```python
from build123d import *

# Parameters (mm, degrees)
SKETCH_2_R          = 11
CUT_EXTRUDE_1_DEPTH = 2
CUT_EXTRUDE_2_REACH = 196.342
SKETCH_3_R          = 5.5
SKETCH_4_R          = 5
CUT_EXTRUDE_3_DEPTH = 46


with BuildPart() as part:
    # 草图1 → 旋转1 (revolve)
    with BuildSketch(Plane.XY, mode=Mode.PRIVATE) as revolve_1_sk:
        with BuildLine():
            Line((65, 35), (57.5, 35))
            Line((57.5, 35), (57.5, 60))
            Line((57.5, 60), (100, 60))
            Line((100, 60), (100, 0))
            Line((100, 0), (130, 0))
            Line((130, 0), (130, -40))
            Line((130, -40), (87.5, -40))
            ThreePointArc((87.5, -40), (80.428932188, -42.928932188), (77.5, -50))
            Line((77.5, -50), (77.5, -65))
            Line((77.5, -65), (65, -65))
            Line((65, -65), (65, 35))
        make_face()
    revolve(revolve_1_sk.sketch.rotate(Axis((0, 133.6875, 0), (0, -1, 0)), 90), axis=Axis((0, 133.6875, 0), (0, -1, 0)))

    # 草图2 → 切除-拉伸1 (cut)
    with BuildSketch(Plane(origin=(0, 0, 0), x_dir=(1, 0, 0), z_dir=(0, 1, 0))):
        with Locations(Location((115, 0, 0), (0, 0, 270))):
            Circle(SKETCH_2_R)
        with Locations(Location((81.317279836, -81.317279836, 0), (0, 0, 270))):
            Circle(SKETCH_2_R)
        with Locations(Location((0, -115, 0), (0, 0, 270))):
            Circle(SKETCH_2_R)
        with Locations(Location((-81.317279836, -81.317279836, 0), (0, 0, 270))):
            Circle(SKETCH_2_R)
        with Locations(Location((-115, 0, 0), (0, 0, 270))):
            Circle(SKETCH_2_R)
        with Locations(Location((-81.317279836, 81.317279836, 0), (0, 0, 270))):
            Circle(SKETCH_2_R)
        with Locations(Location((0, 115, 0), (0, 0, 270))):
            Circle(SKETCH_2_R)
        with Locations(Location((81.317279836, 81.317279836, 0), (0, 0, 270))):
            Circle(SKETCH_2_R)
    extrude(amount=-CUT_EXTRUDE_1_DEPTH, mode=Mode.SUBTRACT)

    # 草图3 → 切除-拉伸2 (cut, up to next)
    with BuildSketch(Plane(origin=(0, -2, 0), x_dir=(1, 0, 0), z_dir=(0, 1, 0)), mode=Mode.PRIVATE) as cut_extrude_2_sk1:
        with Locations(Location((81.317279836, 81.317279836, 0), (0, 0, 270))):
            Circle(SKETCH_3_R)
    cut_extrude_2_tool1 = extrude(cut_extrude_2_sk1.sketch, amount=-CUT_EXTRUDE_2_REACH, mode=Mode.PRIVATE) & part.part
    # 草图3 → 切除-拉伸2 (cut, up to next)
    with BuildSketch(Plane(origin=(0, -2, 0), x_dir=(1, 0, 0), z_dir=(0, 1, 0)), mode=Mode.PRIVATE) as cut_extrude_2_sk2:
        with Locations(Location((115, 0, 0), (0, 0, 270))):
            Circle(SKETCH_3_R)
    cut_extrude_2_tool2 = extrude(cut_extrude_2_sk2.sketch, amount=-CUT_EXTRUDE_2_REACH, mode=Mode.PRIVATE) & part.part
    # 草图3 → 切除-拉伸2 (cut, up to next)
    with BuildSketch(Plane(origin=(0, -2, 0), x_dir=(1, 0, 0), z_dir=(0, 1, 0)), mode=Mode.PRIVATE) as cut_extrude_2_sk3:
        with Locations(Location((81.317279836, -81.317279836, 0), (0, 0, 270))):
            Circle(SKETCH_3_R)
    cut_extrude_2_tool3 = extrude(cut_extrude_2_sk3.sketch, amount=-CUT_EXTRUDE_2_REACH, mode=Mode.PRIVATE) & part.part
    # 草图3 → 切除-拉伸2 (cut, up to next)
    with BuildSketch(Plane(origin=(0, -2, 0), x_dir=(1, 0, 0), z_dir=(0, 1, 0)), mode=Mode.PRIVATE) as cut_extrude_2_sk4:
        with Locations(Location((0, -115, 0), (0, 0, 270))):
            Circle(SKETCH_3_R)
    cut_extrude_2_tool4 = extrude(cut_extrude_2_sk4.sketch, amount=-CUT_EXTRUDE_2_REACH, mode=Mode.PRIVATE) & part.part
    # 草图3 → 切除-拉伸2 (cut, up to next)
    with BuildSketch(Plane(origin=(0, -2, 0), x_dir=(1, 0, 0), z_dir=(0, 1, 0)), mode=Mode.PRIVATE) as cut_extrude_2_sk5:
        with Locations(Location((-81.317279836, -81.317279836, 0), (0, 0, 270))):
            Circle(SKETCH_3_R)
    cut_extrude_2_tool5 = extrude(cut_extrude_2_sk5.sketch, amount=-CUT_EXTRUDE_2_REACH, mode=Mode.PRIVATE) & part.part
    # 草图3 → 切除-拉伸2 (cut, up to next)
    with BuildSketch(Plane(origin=(0, -2, 0), x_dir=(1, 0, 0), z_dir=(0, 1, 0)), mode=Mode.PRIVATE) as cut_extrude_2_sk6:
        with Locations(Location((-115, 0, 0), (0, 0, 270))):
            Circle(SKETCH_3_R)
    cut_extrude_2_tool6 = extrude(cut_extrude_2_sk6.sketch, amount=-CUT_EXTRUDE_2_REACH, mode=Mode.PRIVATE) & part.part
    # 草图3 → 切除-拉伸2 (cut, up to next)
    with BuildSketch(Plane(origin=(0, -2, 0), x_dir=(1, 0, 0), z_dir=(0, 1, 0)), mode=Mode.PRIVATE) as cut_extrude_2_sk7:
        with Locations(Location((-81.317279836, 81.317279836, 0), (0, 0, 270))):
            Circle(SKETCH_3_R)
    cut_extrude_2_tool7 = extrude(cut_extrude_2_sk7.sketch, amount=-CUT_EXTRUDE_2_REACH, mode=Mode.PRIVATE) & part.part
    # 草图3 → 切除-拉伸2 (cut, up to next)
    with BuildSketch(Plane(origin=(0, -2, 0), x_dir=(1, 0, 0), z_dir=(0, 1, 0)), mode=Mode.PRIVATE) as cut_extrude_2_sk8:
        with Locations(Location((0, 115, 0), (0, 0, 270))):
            Circle(SKETCH_3_R)
    cut_extrude_2_tool8 = extrude(cut_extrude_2_sk8.sketch, amount=-CUT_EXTRUDE_2_REACH, mode=Mode.PRIVATE) & part.part
    add(cut_extrude_2_tool1.solids().sort_by_distance((81.31728, -2, -81.31728))[0], mode=Mode.SUBTRACT)
    add(cut_extrude_2_tool2.solids().sort_by_distance((115, -2, 0))[0], mode=Mode.SUBTRACT)
    add(cut_extrude_2_tool3.solids().sort_by_distance((81.31728, -2, 81.31728))[0], mode=Mode.SUBTRACT)
    add(cut_extrude_2_tool4.solids().sort_by_distance((0, -2, 115))[0], mode=Mode.SUBTRACT)
    add(cut_extrude_2_tool5.solids().sort_by_distance((-81.31728, -2, 81.31728))[0], mode=Mode.SUBTRACT)
    add(cut_extrude_2_tool6.solids().sort_by_distance((-115, -2, 0))[0], mode=Mode.SUBTRACT)
    add(cut_extrude_2_tool7.solids().sort_by_distance((-81.31728, -2, -81.31728))[0], mode=Mode.SUBTRACT)
    add(cut_extrude_2_tool8.solids().sort_by_distance((0, -2, -115))[0], mode=Mode.SUBTRACT)

    # 草图4 → 切除-拉伸3 (cut)
    with BuildSketch(Plane(origin=(0, 60, 0), x_dir=(1, 0, 0), z_dir=(0, 1, 0))):
        with Locations(Location((80, 0, 0), (0, 0, 270))):
            Circle(SKETCH_4_R)
        with Locations(Location((56.568542495, -56.568542495, 0), (0, 0, 270))):
            Circle(SKETCH_4_R)
        with Locations(Location((0, -80, 0), (0, 0, 270))):
            Circle(SKETCH_4_R)
        with Locations(Location((-56.568542495, -56.568542495, 0), (0, 0, 270))):
            Circle(SKETCH_4_R)
        with Locations(Location((-80, 0, 0), (0, 0, 270))):
            Circle(SKETCH_4_R)
        with Locations(Location((-56.568542495, 56.568542495, 0), (0, 0, 270))):
            Circle(SKETCH_4_R)
        with Locations(Location((0, 80, 0), (0, 0, 270))):
            Circle(SKETCH_4_R)
        with Locations(Location((56.568542495, 56.568542495, 0), (0, 0, 270))):
            Circle(SKETCH_4_R)
    extrude(amount=-CUT_EXTRUDE_3_DEPTH, mode=Mode.SUBTRACT)


solid = part.part
```
The model under review builds one solid part; all positions refer to its coordinate system, in mm. A direction names the side the tool comes from. Round coordinates to 2 decimals unless told otherwise and drop trailing zeros. Write each loop counter-clockwise with the first axis right and the second up, starting at its lowest first coordinate (ties: lowest second). Pieces come first, ordered by that corner, then holes.
(1) We need section C-C on y = -54. Give the boundary of the cut face in (x, z), and give its area (3 significant figures).
(2) We need section D-D on z = -115. Give the boundary of the cut face in (x, y), and give its area (3 significant figures).
(3) Mouldability with a two-part tool opening along Z and no side actions: class faces 1 (the cylindrical face through (-39.048, -20.28, 123.997)), 2 (the flat face through (43, 60, -43)), 3 (the flat face through (-84, -2, 76)) as +Z half, -Z half, draft (parallel to the pull), parting line (faces both ways), or undercut.
(4) Wall thickness on L1, parallel to X at y = -51.5, z = -0.5; L2, parallel to X at y = -42.5, z = -19; L3, parallel to Y at x = -63, z = 101: over which ranges is each line inside the solid? List them lowest first.
(5) Insertion check: pin 1 (2 mm diameter, centred on x = -101.5, z = -8.5, fed in from -Y); pin 2 (6 mm diameter, centred on x = -56.57, z = 56.57, fed in from -Y); pin 3 (12 mm diameter, centred on x = -42, y = 35, fed in from +Z); pin 4 (17.5 mm diameter, centred on x = 81.32, z = 81.32, fed in from +Y). Each pin has a flat end and moves straight along its axis. Give the tip position at first contact, or say it passes through.
(6) We need section B-B on z = 0. Give the number of separate pieces and of enclosed holes in the cut face, and give its area (3 significant figures).
(7) We need section A-A on x = 115. Give the boundary of the cut face in (y, z), and give its area (3 significant figures).
(8) Machinability: for faces 4 (the cylindrical face through (61.526, 37.322, 55.918)), 5 (the cylindrical face through (-109.547, -20.734, -0.716)), 6 (the flat face through (-88, -40, -2)), which of the approach directions +Z, -Z, +X, -X, +Y, -Y give a long, thin tool a straight path to every point of the face, cutting with its end or side? Answer none if there is none.
Findings below:
1. outline: circle Ø155 at (0, 0); hole circle Ø130 at (0, 0)
1. area: 5,600 mm2
2. outline: (-60.62, -40) - (-5.5, -40) - (-5.5, -2) - (-11, -2) - (-11, 0) - (-60.62, 0) - close; (5.5, -40) - (60.62, -40) - (60.62, 0) - (11, 0) - (11, -2) - (5.5, -2) - close
2. area: 4,390 mm2
3. face 1: parting line
3. face 2: draft
3. face 3: undercut
4. L1: x = -77.5 to -65, 65 to 77.5
4. L2: x = -78.62 to -62.16, 62.16 to 78.62
4. L3: y = -40 to 0
5. pin 1: stops at y = -40
5. pin 2: stops at y = -65
5. pin 3: stops at z = 93.3
5. pin 4: stops at y = -2
6. separate pieces: 4
6. enclosed holes: 0
6. area: 8,600 mm2
7. outline: (-40, -60.62) - (0, -60.62) - (0, -11) - (-2, -11) - (-2, -5.5) - (-40, -5.5) - close; (-40, 5.5) - (-2, 5.5) - (-2, 11) - (0, 11) - (0, 60.62) - (-40, 60.62) - close
7. area: 4,390 mm2
8. face 4: +Y
8. face 5: +Y, -Y
8. face 6: -Y
